Could you check a few things on this model? Use its own coordinates, in mm. Face numbers are marked on the shaded views. A direction names the side the tool comes from. Give positions to 0.01 mm unless a question says otherwise; leave off trailing zeros. Write each loop counter-clockwise with the first axis right and the second up, starting at its lowest first coordinate (ties: lowest second). Pieces come first, ordered by that corner, then holes. Notation, with made-up numbers: (56.5, 23.5) - (70.5, 23.5) arc R30 cw to (70.5, 61.5) - close; hole circle Ø4 at (85, 63). An arc over 180 degrees is marked (long way). Answer in a Markdown table with one row per item.
from build123d import *

# Parameters (mm, degrees)
BOSS_EXTRUDE1_DEPTH = 80
SKETCH2_W           = 5
SKETCH2_H           = 80
BOSS_EXTRUDE2_DEPTH = 15
SKETCH3_W           = 5
SKETCH3_H           = 80
BOSS_EXTRUDE3_DEPTH = 15
FILLET1_R           = 10
FILLET2_R           = 5
SKETCH4_W           = 60
SKETCH4_H           = 5
BOSS_EXTRUDE4_DEPTH = 15
SKETCH5_W           = 60
SKETCH5_H           = 5
BOSS_EXTRUDE5_DEPTH = 25
FILLET3_R           = 5
FILLET4_R           = 10
SKETCH6_R           = 1.6
CUT_EXTRUDE1_DEPTH  = 10
FILLET5_R           = 10
SKETCH7_R           = 1.6
CUT_EXTRUDE2_DEPTH  = 188.149672722
SKETCH8_R           = 1.6
CUT_EXTRUDE3_DEPTH  = 184.439363278


with BuildPart() as part:
    # Sketch1 → Boss-Extrude1 (new body)
    with BuildSketch(Plane(origin=(0, 0, 0), x_dir=(1, 0, 0), z_dir=(0, 1, 0))):
        Polygon((0, 0), (0, 134.306122449), (5, 134.306122449), (5, -0.693877551), (75, -0.693877551), (75, 134.306122449), (80, 134.306122449), (80, -5.693877551), (35.857142857, -5.693877551), (0, -5.693877551), align=None)
    extrude(amount=BOSS_EXTRUDE1_DEPTH)

    # Sketch2 → Boss-Extrude2 (add)
    with BuildSketch(Plane(origin=(80, 0, 0), x_dir=(0, 0, -1), z_dir=(1, 0, 0))):
        with Locations((131.806122449, 40)):
            Rectangle(SKETCH2_W, SKETCH2_H)
    extrude(amount=BOSS_EXTRUDE2_DEPTH)

    # Sketch3 → Boss-Extrude3 (add)
    with BuildSketch(Plane.ZY):
        with Locations((-131.806122449, 40)):
            Rectangle(SKETCH3_W, SKETCH3_H)
    extrude(amount=BOSS_EXTRUDE3_DEPTH)

    # Fillet1
    fillet1_edges = [part.edges().sort_by_distance(p)[0] for p in [
        (5, 40, -134.306122449),
        (75, 40, -134.306122449),
        (80, 40, 5.693877551),
        (0, 40, 5.693877551),
    ]]
    fillet(fillet1_edges, radius=FILLET1_R)

    # Fillet2
    fillet2_edges = [part.edges().sort_by_distance(p)[0] for p in [
        (5, 40, 0.693877551),
        (75, 40, 0.693877551),
        (80, 40, -129.306122449),
        (0, 40, -129.306122449),
    ]]
    fillet(fillet2_edges, radius=FILLET2_R)

    # Sketch4 → Boss-Extrude4 (add)
    with BuildSketch(Plane.XZ):
        with Locations((40, 3.193877551)):
            Rectangle(SKETCH4_W, SKETCH4_H)
    extrude(amount=BOSS_EXTRUDE4_DEPTH)

    # Sketch5 → Boss-Extrude5 (add)
    with BuildSketch(Plane(origin=(0, 0, 0.693877551), x_dir=(-1, 0, 0), z_dir=(0, 0, -1))):
        with Locations((-40, -12.5)):
            Rectangle(SKETCH5_W, SKETCH5_H)
    extrude(amount=BOSS_EXTRUDE5_DEPTH)

    # Fillet3
    fillet3_edges = [part.edges().sort_by_distance(p)[0] for p in [
        (40, -10, 0.693877551),
    ]]
    fillet(fillet3_edges, radius=FILLET3_R)

    # Fillet4
    fillet4_edges = [part.edges().sort_by_distance(p)[0] for p in [
        (40, -15, 5.693877551),
    ]]
    fillet(fillet4_edges, radius=FILLET4_R)

    # Sketch6 → Cut-Extrude1 (cut)
    with BuildSketch(Plane.XZ.offset(15)):
        with Locations(Location((17.5, -16.306122449, 0), (0, 0, 270))):
            Circle(SKETCH6_R)
        with Locations(Location((62.5, -16.306122449, 0), (0, 0, 270))):
            Circle(SKETCH6_R)
    extrude(amount=-CUT_EXTRUDE1_DEPTH, mode=Mode.SUBTRACT)

    # Fillet5
    fillet5_edges = [part.edges().sort_by_distance(p)[0] for p in [
        (70, -12.5, -24.306122449),
        (10, -12.5, -24.306122449),
    ]]
    fillet(fillet5_edges, radius=FILLET5_R)

    # Sketch7 → Cut-Extrude2 (cut, through all)
    with BuildSketch(Plane.XY.offset(5.693877551)):
        with Locations((22, 64)):
            Circle(SKETCH7_R)
        with Locations((58, 64)):
            Circle(SKETCH7_R)
        with Locations((58, 16)):
            Circle(SKETCH7_R)
        with Locations((22, 16)):
            Circle(SKETCH7_R)
    extrude(amount=-CUT_EXTRUDE2_DEPTH, mode=Mode.SUBTRACT)

    # Sketch8 → Cut-Extrude3 (cut, through all)
    with BuildSketch(Plane.XY.offset(-129.306122449)):
        with Locations((-10, 70)):
            Circle(SKETCH8_R)
        with Locations((-10, 40)):
            Circle(SKETCH8_R)
        with Locations((-10, 10)):
            Circle(SKETCH8_R)
        with Locations((90, 70)):
            Circle(SKETCH8_R)
        with Locations((90, 40)):
            Circle(SKETCH8_R)
        with Locations((90, 10)):
            Circle(SKETCH8_R)
    extrude(amount=-CUT_EXTRUDE3_DEPTH, mode=Mode.SUBTRACT)


solid = part.part
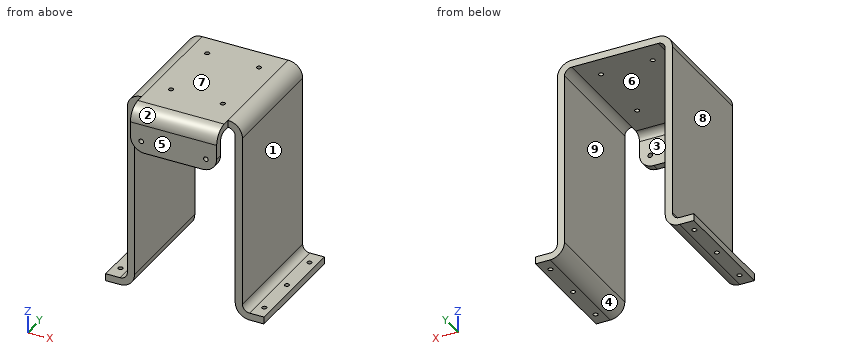
1) Imagine slicing it at A-A (z = -35). List the corners of the cut face in (x, y) for me, then the cut area to 3 significant figures.
Check values:
| item | result |
|---|---|
| outline | (0, 0) - (5, 0) - (5, 80) - (0, 80) - close; (75, 0) - (80, 0) - (80, 80) - (75, 80) - close |
| area | 800 mm2 |
2) We'd pull the mould along X, two halves only. Please class the marked faces 6, 7, 8 and 9: +X half, -X half, draft (parallel to the pull), parting line (faces both ways), or undercut.
Check values:
| item | result |
|---|---|
| face 6 | undercut |
| face 7 | draft |
| face 8 | -X half |
| face 9 | undercut |
3) Imagine slicing it at C-C (y = 24). List the corners of the cut face in (x, z) for me.
Check values:
| item | result |
|---|---|
| outline | (-15, -134.31) - (-5, -134.31) arc R10 ccw to (5, -124.31) - (5, -4.31) arc R5 cw to (10, 0.69) - (70, 0.69) arc R5 cw to (75, -4.31) - (75, -124.31) arc R10 ccw to (85, -134.31) - (95, -134.31) - (95, -129.31) - (85, -129.31) arc R5 cw to (80, -124.31) - (80, -4.31) arc R10 ccw to (70, 5.69) - (10, 5.69) arc R10 ccw to (0, -4.31) - (0, -124.31) arc R5 cw to (-5, -129.31) - (-15, -129.31) - close |
4) Imagine slicing it at D-D (z = -9.5). List the corners of the cut face in (x, y) for me, then the cut area to 3 significant figures.
Check values:
| item | result |
|---|---|
| outline | (0, 0) - (5, 0) - (5, 80) - (0, 80) - close; (10, -15) - (70, -15) - (70, -10) - (10, -10) - close; (75, 0) - (80, 0) - (80, 80) - (75, 80) - close |
| area | 1,100 mm2 |
5) If I drill on line 1 (Y direction, x = 90, z = -130); line 2 (X direction, y = 63.5, z = -22.5); line 3 (X direction, y = 70, z = -130.7), over which ranges is the centre line in solid material (lowest first)?
Check values:
| item | result |
|---|---|
| line 1 | y = 0 to 8.4, 11.6 to 38.4, 41.6 to 68.4, 71.6 to 80 |
| line 2 | x = 0 to 5, 75 to 80 |
| line 3 | x = -15 to -11.6, -8.4 to 2.69, 77.31 to 88.4, 91.6 to 95 |
6) Will these pins go through, and if not, where does the flat tip stop? P1, Ø10, axis at x = 52, z = -18.5, coming from the +Y side; P2, Ø5, axis at x = 38, y = 38, coming from the -Z side; P3, Ø6, axis at y = 20, z = -96, coming from the +X side.
Check values:
| item | result |
|---|---|
| P1 | stops at y = -10 |
| P2 | stops at z = 0.69 |
| P3 | stops at x = 80 |
7) Imagine slicing it at B-B (x = 36.5). List the corners of the cut face in (y, z) for me, then the cut area to 3 significant figures.
Check values:
| item | result |
|---|---|
| outline | (-15, -24.31) - (-10, -24.31) - (-10, -4.31) arc R5 cw to (-5, 0.69) - (80, 0.69) - (80, 5.69) - (-5, 5.69) arc R10 ccw to (-15, -4.31) - close |
| area | 584 mm2 |
8) On a 3-axis mill with a long thin cutter (end or side, diameter ignored), from which of +Z, -Z, +X, -X, +Y, -Y can I reach the whole of each face in a straight line? I mean the marked faces 1, 2, 3, 4 and 5. Say none if no direction works.
Check values:
| item | result |
|---|---|
| face 1 | +Z, +X, +Y, -Y |
| face 2 | +Z, +X, -X, -Y |
| face 3 | -Z, +X, -X, +Y |
| face 4 | -Z, +Y, -Y |
| face 5 | +Z, -Z, +X, -X, -Y |
